Design review of the part built by this model. Coordinates are the model's own, in mm. Coordinates: 2 decimals unless noted, no trailing zeros. Loops run counter-clockwise (first coordinate to the right, second up) from the corner with the lowest first, then second, coordinate; pieces in that order, holes last. Notation, with made-up numbers: (13, 33) -> (69, 33) arc R28 cw to (69, 72) -> close; hole circle Ø11 at (52.25, 24). An arc over 180 degrees is marked (long way). Answer in a Markdown table with one row per item.
```python
from build123d import *

# Parameters (mm, degrees)
SKETCH1_W           = 120
SKETCH1_H           = 1000
BOSS_EXTRUDE1_DEPTH = 300
CHAMFER1_SIZE       = 50


with BuildPart() as part:
    # Sketch1 → Boss-Extrude1 (new body)
    with BuildSketch(Plane.XY):
        Rectangle(SKETCH1_W, SKETCH1_H)
    extrude(amount=BOSS_EXTRUDE1_DEPTH)

    # Chamfer1
    chamfer1_edges = [part.edges().sort_by_distance(p)[0] for p in [
        (60, 0, 300),
    ]]
    chamfer(chamfer1_edges, length=CHAMFER1_SIZE)


solid = part.part
```
(1) To check wall thickness, follow probe 1 along Z at (x, y) = (22, -362); probe 2 along Z at (x, y) = (27.5, 120); probe 3 along X at (y, z) = (247, 285). State the ranges of each line that lie inside material, in increasing order.
Evaluation:
| item | result |
|---|---|
| probe 1 | z = 0 to 288 |
| probe 2 | z = 0 to 282.5 |
| probe 3 | x = -60 to 25 |
(2) Take a section at B-B on x = 24.5. Give the boundary of the cut face in (y, z).
Evaluation:
| item | result |
|---|---|
| outline | (-500, 0) -> (500, 0) -> (500, 285.5) -> (-500, 285.5) -> close |
(3) Take a section at C-C on z = 278.5. Give the boundary of the cut face in (x, y), and give its area (3 significant figures).
Evaluation:
| item | result |
|---|---|
| outline | (-60, -500) -> (31.5, -500) -> (31.5, 500) -> (-60, 500) -> close |
| area | 91,500 mm² |
(4) For pin 1 (8 mm diameter, centred on x = 39.5, y = -54.5, fed in from +Z); pin 2 (1 mm diameter, centred on x = 26.5, y = -173, fed in from -Z), all flat-tipped, find the tip position at first contact; note any pin that passes through.
Evaluation:
| item | result |
|---|---|
| pin 1 | stops at z = 274.5 |
| pin 2 | stops at z = 0 |
(5) Take a section at A-A on y = 149. Give the boundary of the cut face in (x, z).
Evaluation:
| item | result |
|---|---|
| outline | (-60, 0) -> (60, 0) -> (60, 250) -> (10, 300) -> (-60, 300) -> close |
